Geometry check sheet. Reference: the model listing, model coordinates, mm. A direction names the side the tool comes from. Coordinates: 2 decimals unless noted, no trailing zeros. Write each loop counter-clockwise with the first axis right and the second up, starting at its lowest first coordinate (ties: lowest second). Pieces come first, ordered by that corner, then holes. Notation, with made-up numbers: M -31.75,0 L 13.25,0 A29 cw 13.25,22 Z; hole C -10,63.25 d3. An arc over 180 degrees is marked long. Put each result on its own line as item: value. Start each with the question number.
1) Gauge pin test, flat ends, axial feed: pin 1 (12 mm diameter, centred on y = -1, z = 13.5, fed in from +X); pin 2 (1 mm diameter, centred on y = -1, z = 3.5, fed in from -X); pin 3 (1.5 mm diameter, centred on x = 26.5, z = 11.5, fed in from +Y). Record the tip position at first contact, or that the pin passes through.
2) Cross-section at D-D on y = 83. Record the cut outline in (x, z), plus the area to 3 significant figures.
3) Cross-section at C-C on y = 0. Record the cut outline in (x, z), plus the area to 3 significant figures.
4) Mould release check, pull along X, two halves, no side actions. Record for faces 4 (the flat face through (-19, 93, 6)), 5 (the cylindrical face through (83.137, -4.471, 9.86)), 6 (the flat face through (-54, -36, 20)): released by +X, released by -X, zero draft, split by the parting line, or undercut.
5) Cross-section at A-A on x = 0. Record the cut outline in (y, z).
6) Scan lines: line 1 along Y through (x, z) = (0, 1.55); line 2 along Y through (x, z) = (0, 10); line 3 along Y through (x, z) = (3, 1.75). Record each from-to range of solid material in increasing order.
7) Cross-section at B-B on z = 3. Record the cut outline in (x, y).
8) Set-up check for faces 1 (the flat face through (-1, 31, 20)), 2 (the flat face through (-19, -33, 14)), 3 (the cylindrical face through (62, 10.48, 3.04)): record each of +Z, -Z, +X, -X, +Y, -Y from which the full face is reachable in a straight line by a thin tool's end or side.
from build123d import *

# Parameters (mm, degrees)
SKETCH1_R           = 90
SKETCH1_R_2         = 30
BOSS_EXTRUDE1_DEPTH = 20
SKETCH2_R           = 85
SKETCH2_R_2         = 65
CUT_EXTRUDE1_DEPTH  = 6
CUT_EXTRUDE2_START  = -6
SKETCH3_R           = 85
SKETCH3_R_2         = 65
CUT_EXTRUDE2_DEPTH  = 6


with BuildPart() as part:
    # Sketch1 → Boss-Extrude1 (new body)
    with BuildSketch(Plane.XY):
        with Locations((0, 30)):
            Circle(SKETCH1_R)
        Circle(SKETCH1_R_2, mode=Mode.SUBTRACT)
    extrude(amount=BOSS_EXTRUDE1_DEPTH)

    # Sketch2 → Cut-Extrude1 (cut)
    with BuildSketch(Plane.XY.offset(20)):
        with Locations((0, 30)):
            Circle(SKETCH2_R)
        with Locations((0, 30)):
            Circle(SKETCH2_R_2, mode=Mode.SUBTRACT)
    extrude(amount=-CUT_EXTRUDE1_DEPTH, mode=Mode.SUBTRACT)

    # Sketch3 → Cut-Extrude2 (cut)
    with BuildSketch(Plane(origin=(0, 0, 0), x_dir=(-1, 0, 0), z_dir=(0, 0, -1)).offset(CUT_EXTRUDE2_START)):
        with Locations(Location((0, 30, 0), (0, 0, 180))):
            Circle(SKETCH3_R)
        with Locations(Location((0, 30, 0), (0, 0, 180))):
            Circle(SKETCH3_R_2, mode=Mode.SUBTRACT)
    extrude(amount=CUT_EXTRUDE2_DEPTH, mode=Mode.SUBTRACT)


solid = part.part
Answer key:
1. pin 1: stops at x = 86.46
1. pin 2: stops at x = -84.67
1. pin 3: stops at y = 116.24
2. outline: M -72.74,0 L -66.45,0 L -66.45,6 L -37.63,6 L -37.63,0 L 37.63,0 L 37.63,6 L 66.45,6 L 66.45,0 L 72.74,0 L 72.74,20 L 66.45,20 L 66.45,14 L 37.63,14 L 37.63,20 L -37.63,20 L -37.63,14 L -66.45,14 L -66.45,20 L -72.74,20 Z
2. area: 2,220 mm²
3. outline: M -84.85,0 L -79.53,0 L -79.53,6 L -57.66,6 L -57.66,0 L -30,0 L -30,20 L -57.66,20 L -57.66,14 L -79.53,14 L -79.53,20 L -84.85,20 Z; M 30,0 L 57.66,0 L 57.66,6 L 79.53,6 L 79.53,0 L 84.85,0 L 84.85,20 L 79.53,20 L 79.53,14 L 57.66,14 L 57.66,20 L 30,20 Z
3. area: 1,670 mm²
4. face 4: undercut
4. face 5: split by the parting line
4. face 6: zero draft
5. outline: M -60,0 L -55,0 L -55,6 L -35,6 L -35,0 L -30,0 L -30,20 L -35,20 L -35,14 L -55,14 L -55,20 L -60,20 Z; M 30,0 L 95,0 L 95,6 L 115,6 L 115,0 L 120,0 L 120,20 L 115,20 L 115,14 L 95,14 L 95,20 L 30,20 Z
6. line 1: y = -60 to -55, -35 to -30, 30 to 95, 115 to 120
6. line 2: y = -60 to -30, 30 to 120
6. line 3: y = -59.95 to -54.95, -34.93 to -29.85, 29.85 to 94.93, 114.95 to 119.95
7. outline: C 0,30 d180; C 0,30 d130; hole C 0,30 d170; hole C 0,0 d60
8. face 1: +Z, +X, -X, +Y, -Y
8. face 2: +Z
8. face 3: -Z
